Job drawing, mm, ordinate dimensions from the low corner. One solid piece. Round coordinates to 2 decimals unless told otherwise and drop trailing zeros. Write each loop counter-clockwise with the first axis right and the second up, starting at its lowest first coordinate (ties: lowest second). Pieces come first, ordered by that corner, then holes. Notation, with made-up numbers: M 14,46 L 70,46 A23 cw 70,71 Z; hole C 16,68.25 d9. An arc over 180 degrees is marked long. Answer as a JSON object with one key per item and string values. Group by question number.
1. Two-plate mould, pull along X, no slides. Class the marked faces 1, 2, 3 and 4: +X half, -X half, draft (parallel to the pull), parting line (faces both ways), or undercut.
2. Band-saw the part on B-B, the plane y = 10. Write the cut outline in (x, z), plus the area to 3 significant figures.
3. Drop a flat-ended pin along its axis: pin 1 (1.5 mm diameter, centred on y = 10.5, z = 1.5, fed in from -X). Give the stop position or say it passes through.
4. Drill centre lines: line 1 (Y direction, x = 20, z = 2.25); line 2 (X direction, y = 7.75, z = 2.25); line 3 (X direction, y = 8.25, z = 2). Where is each one in solid material? Low to high. Write a range as from..to.
5. Band-saw the part on A-A, the plane x = 20. Write the cut outline in (y, z), plus the area to 3 significant figures.
6. Band-saw the part on C-C, the plane z = 1.55. Write the cut outline in (x, y).
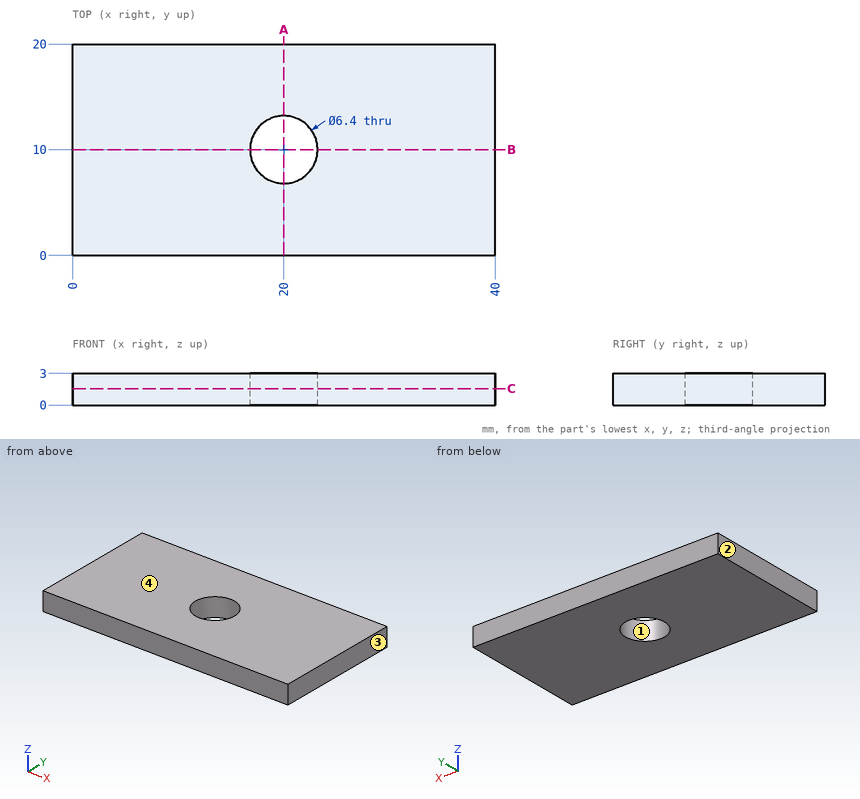
Worked answers:
{
 "1": {"face 1": "undercut", "face 2": "-X half", "face 3": "+X half", "face 4": "draft"},
 "2": {"outline": "M 0,0 L 16.8,0 L 16.8,3 L 0,3 Z; M 23.2,0 L 40,0 L 40,3 L 23.2,3 Z", "area": "101 mm^2"},
 "3": {"pin 1": "stops at x = 0"},
 "4": {"line 1": "y = 0..6.8, 13.2..20", "line 2": "x = 0..17.72, 22.28..40", "line 3": "x = 0..17.32, 22.68..40"},
 "5": {"outline": "M 0,0 L 6.8,0 L 6.8,3 L 0,3 Z; M 13.2,0 L 20,0 L 20,3 L 13.2,3 Z", "area": "40.8 mm^2"},
 "6": {"outline": "M 0,0 L 40,0 L 40,20 L 0,20 Z; hole C 20,10 d6.4"}
}
